Input: part model. Units: mm. Frame: model coordinates. Round coordinates to 2 decimals unless told otherwise and drop trailing zeros. Loops run counter-clockwise (first coordinate to the right, second up) from the corner with the lowest first, then second, coordinate; pieces in that order, holes last. Notation, with made-up numbers: (53, 57.5) -> (60, 57.5) arc R11 ccw to (60, 66.5) -> close; hole circle Ø5 at (-20, -30). An arc over 180 degrees is marked (long way). Answer as a JSON object with one key per item and string values.
```python
from build123d import *

# Parameters (mm, degrees)
SWEEP_THIN1_PROFILE_R   = 15
SWEEP_THIN1_PROFILE_R_2 = 13


with BuildPart() as part:
    # Sweep-Thin1: sweep along a curve in space
    with BuildLine() as sweep_thin1_path:
        Line((19403.083026604, -840, -3659.86490803), (19403.083026604, -807.464377163, -3659.86490803))
        ThreePointArc((19403.083026604, -807.464377163, -3659.86490803), (19403.083026604, -790.016622217, -3659.484196663), (19403.083026604, -772.602080064, -3658.342787267))
        Line((19403.083026604, -772.602080064, -3658.342787267), (19403.083026604, 116.074565195, -3580.593655266))
        ThreePointArc((19403.083026604, 116.074565195, -3580.593655266), (19403.083026604, 133.489107348, -3579.45224587), (19403.083026604, 150.936862294, -3579.071534503))
        Line((19403.083026604, 150.936862294, -3579.071534503), (19403.083026604, 213.472485131, -3579.071534503))
    # Sweep-Thin1 profile (on start of the path) → Sweep-Thin1 (sweep)
    with BuildSketch(Plane(origin=(19403.083026604, -840, -3659.86490803), x_dir=(0, 0, 1), z_dir=(0, 1, 0))):
        Circle(SWEEP_THIN1_PROFILE_R)
        Circle(SWEEP_THIN1_PROFILE_R_2, mode=Mode.SUBTRACT)
    sweep(path=sweep_thin1_path.line)


solid = part.part
```
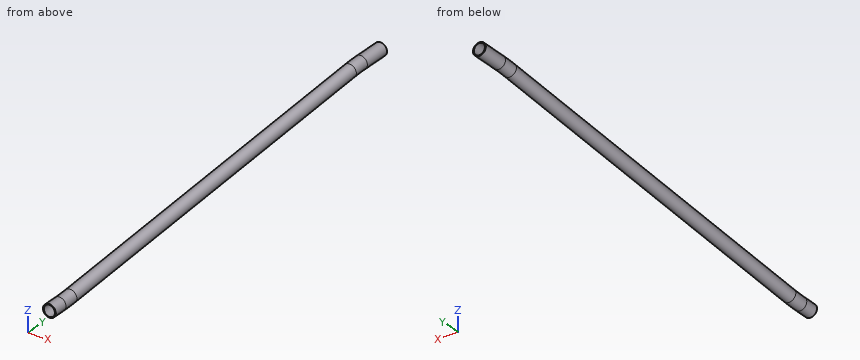
1) Section A-A, the plane x = 19398.5. Output: boundary loops of the cut face in (y, z), plus the area to 3 significant figures.
Output:
{"outline": "(-840, -3674.15) -> (-807.46, -3674.15) arc R414.28 ccw to (-771.36, -3672.57) -> (117.32, -3594.82) arc R385.72 cw to (150.94, -3593.35) -> (213.47, -3593.35) -> (213.47, -3591.24) -> (150.94, -3591.24) arc R387.83 ccw to (117.13, -3592.71) -> (-771.54, -3670.46) arc R412.17 cw to (-807.46, -3672.03) -> (-840, -3672.03) -> close; (-840, -3647.7) -> (-807.46, -3647.7) arc R387.83 ccw to (-773.66, -3646.22) -> (115.01, -3568.47) arc R412.17 cw to (150.94, -3566.91) -> (213.47, -3566.91) -> (213.47, -3564.79) -> (150.94, -3564.79) arc R414.28 ccw to (114.83, -3566.37) -> (-773.85, -3644.11) arc R385.72 cw to (-807.46, -3645.58) -> (-840, -3645.58) -> close", "area": "4,480 mm^2"}
2) Contact query for flat-ended pins moving along their axis: P1, Ø10, axis at x = 19412, y = -717, coming from the -Z side; P2, Ø6, axis at x = 19397, y = -20.5, coming from the -Z side; P3, Ø1, axis at x = 19413.5, y = 56, coming from the +Z side. Output: stop coordinate, or through.
Output:
{"P1": "stops at z = -3668.08", "P2": "stops at z = -3607.33", "P3": "stops at z = -3574.55"}
3) Ray query, probe 1 along Z at (x, y) = (19393.5, 76); probe 2 along Z at (x, y) = (19412.5, -634); probe 3 along X at (y, z) = (-134.5, -3594.5). Return the intervals inside material, ascending.
Output:
{"probe 1": "z = -3595.68 to -3592.92, -3575.28 to -3572.52", "probe 2": "z = -3657.94 to -3655.21, -3637.22 to -3634.5", "probe 3": "x = 19390.39 to 19392.82, 19413.34 to 19415.78"}
